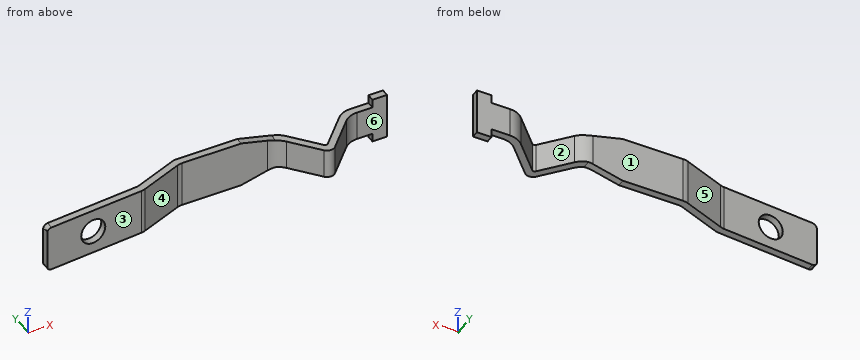
```python
from build123d import *

# Parameters (mm, degrees)
BOSS_EXTRUDE1_DEPTH = 4.75
SKETCH2_OUTSIDE_W   = 89.832
SKETCH2_OUTSIDE_H   = 26.332
SKETCH2_OUTSIDE_R   = 2.6
CUT_EXTRUDE1_DEPTH  = 30


with BuildPart() as part:
    # Sketch1 → Boss-Extrude1 (new, symmetric)
    with BuildSketch(Plane.XY):
        with BuildLine():
            Line((128.472093399, 20.626012941), (135.279511004, 20.626012941))
            Line((135.279511004, 20.626012941), (135.279511004, 19.126012941))
            Line((135.279511004, 19.126012941), (129.116456396, 19.126012941))
            ThreePointArc((129.116456396, 19.126012941), (127.537662704, 18.801255856), (126.215231232, 17.879718181))
            Line((126.215231232, 17.879718181), (120.723107444, 12.093373476))
            ThreePointArc((120.723107444, 12.093373476), (119.592910743, 11.626607721), (118.490782391, 12.156256613))
            Line((118.490782391, 12.156256613), (113.782718692, 17.712029816))
            ThreePointArc((113.782718692, 17.712029816), (112.412732854, 18.755342597), (110.731077047, 19.126012941))
            Line((110.731077047, 19.126012941), (93.127493614, 19.126012941))
            ThreePointArc((93.127493614, 19.126012941), (92.571949476, 19.074126018), (92.035622322, 18.920260082))
            Line((92.035622322, 18.920260082), (83.526071058, 15.595094388))
            ThreePointArc((83.526071058, 15.595094388), (83.117810035, 15.468266897), (82.695666994, 15.400757434))
            Line((82.695666994, 15.400757434), (62.410244618, 13.626012941))
            Line((62.410244618, 13.626012941), (62.279511004, 15.120304988))
            Line((62.279511004, 15.120304988), (82.350355756, 16.876276372))
            ThreePointArc((82.350355756, 16.876276372), (82.772498797, 16.943785835), (83.180759819, 17.070613325))
            Line((83.180759819, 17.070613325), (91.752961452, 20.420260082))
            ThreePointArc((91.752961452, 20.420260082), (92.289288606, 20.574126018), (92.844832744, 20.626012941))
            Line((92.844832744, 20.626012941), (111.42610449, 20.626012941))
            ThreePointArc((111.42610449, 20.626012941), (113.107760296, 20.255342597), (114.477746134, 19.212029816))
            Line((114.477746134, 19.212029816), (119.274777803, 13.551269534))
            ThreePointArc((119.274777803, 13.551269534), (119.64215392, 13.374719903), (120.018886154, 13.530308488))
            Line((120.018886154, 13.530308488), (125.570868236, 19.379718181))
            ThreePointArc((125.570868236, 19.379718181), (126.893299708, 20.301255856), (128.472093399, 20.626012941))
        make_face()
    extrude(amount=BOSS_EXTRUDE1_DEPTH, both=True)

    # Sketch2 outside → Cut-Extrude1 (cut)
    # profile 1 of 2: a face of its own
    with BuildSketch(Plane(origin=(0, 0, 0), x_dir=(1, 0, 0), z_dir=(0, 1, 0))):
        with Locations((98.78, 0)):
            Rectangle(SKETCH2_OUTSIDE_W, SKETCH2_OUTSIDE_H)
        with BuildLine():
            Line((132.279511004, 4.75), (132.279511004, 3))
            Line((132.279511004, 3), (112.256897869, 3))
            Line((112.256897869, 3), (105.256897869, 4.75))
            Line((105.256897869, 4.75), (63.279511004, 4.75))
            ThreePointArc((63.279511004, 4.75), (62.572404223, 4.457106781), (62.279511004, 3.75))
            Line((62.279511004, 3.75), (62.279511004, -3.75))
            ThreePointArc((62.279511004, -3.75), (62.572404223, -4.457106781), (63.279511004, -4.75))
            Line((63.279511004, -4.75), (105.256897869, -4.75))
            Line((105.256897869, -4.75), (112.256897869, -3))
            Line((112.256897869, -3), (132.279511004, -3))
            Line((132.279511004, -3), (132.279511004, -4.75))
            Line((132.279511004, -4.75), (135.279511004, -4.75))
            Line((135.279511004, -4.75), (135.279511004, 4.75))
            Line((135.279511004, 4.75), (132.279511004, 4.75))
        make_face(mode=Mode.SUBTRACT)
    # profile 2 of 2: a face of its own
    with BuildSketch(Plane(origin=(0, 0, 0), x_dir=(1, 0, 0), z_dir=(0, 1, 0))):
        with Locations(Location((72.279511004, 0, 0), (0, 0, 180))):
            Circle(SKETCH2_OUTSIDE_R)
    extrude(amount=CUT_EXTRUDE1_DEPTH, mode=Mode.SUBTRACT)


solid = part.part
```
The listing builds one solid part. Answer for the finished solid, in the listing's coordinates (mm). Face numbers are marked on the shaded views. A direction names the side the tool comes from. Give positions to 0.01 mm unless a question says otherwise; leave off trailing zeros. Order: outer loops, then holes, each group sorted by start corner. A loop starts at its lowest first (then second) coordinate and runs counter-clockwise, first axis right, second up. Notation, with made-up numbers: M -25.5,75.5 L 22.5,75.5 A18 cw 22.5,108.5 Z; hole C -7,77 d4. An arc over 180 degrees is marked long. Put each result on its own line as item: value. Start each with the question number.
Item 1: The part is cut by section B-B, the plane x = 74. Determine the outline of the cut face in (y, z), and give its area (3 significant figures).
Item 2: For a pull along X with two mould halves and no side action, classify the marked faces 4, 5 and 6 as +X half, -X half, draft (parallel to the pull), parting line (faces both ways), or undercut.
Item 3: Which of the six approach directions +Z, -Z, +X, -X, +Y, -Y give full straight-line access (tool end or side, diameter ignored) to the marked faces 1, 2 and 3?
Item 4: Flat-ended cylindrical pins translate along their axes: P1, Ø5, axis at x = 82, y = 17.5, coming from the -Z side; P2, Ø1.5, axis at x = 126.5, z = 1, coming from the +Y side; P3, Ø4.5, axis at x = 126, y = 16.5, coming from the -Z side; P4, Ø3, axis at x = 100, z = 1.5, coming from the -Y side. Find the tip coordinate at first contact, or state that the pin passes through.
Item 5: Find the intervals of material crossed by line 1 along X through (y, z) = (14.5, 0); line 2 along Y through (x, z) = (101, 1.5); line 3 along Z through (x, y) = (131, 19.5), in increasing order.
Item 6: The part is cut by section A-A, the plane z = 0. Determine the outline of the cut face in (x, y).
Item 7: The part is cut by section D-D, the plane x = 124.5. Determine the outline of the cut face in (y, z), and give its area (3 significant figures).
Item 8: The part is cut by section C-C, the plane x = 96.5. Determine the outline of the cut face in (y, z), and give its area (4 significant figures).
Answer key:
1. outline: M 14.64,-4.75 L 16.15,-4.75 L 16.15,-1.95 L 14.64,-1.95 Z; M 14.64,1.95 L 16.15,1.95 L 16.15,4.75 L 14.64,4.75 Z
1. area: 8.43 mm²
2. face 4: undercut
2. face 5: -X half
2. face 6: draft
3. face 1: +Z, -Z, +X, -X, +Y
3. face 2: +Z, -Z, +Y
3. face 3: +Z, -Z, -Y
4. P1: stops at z = -4.75
4. P2: stops at y = 20.43
4. P3: stops at z = -3
4. P4: stops at y = 19.13
5. line 1: x = 62.33 to 69.68, 116.5 to 118.47, 120.94 to 123.01
5. line 2: y = 19.13 to 20.63
5. line 3: z = -3 to 3
6. outline: M 62.28,15.12 L 62.41,13.63 L 69.68,14.26 L 69.68,15.77 Z; M 74.88,14.72 L 82.7,15.4 A3 ccw 83.53,15.6 L 92.04,18.92 A3 cw 93.13,19.13 L 110.73,19.13 A4 cw 113.78,17.71 L 118.49,12.16 A1.5 ccw 120.72,12.09 L 126.22,17.88 A4 cw 129.12,19.13 L 135.28,19.13 L 135.28,20.63 L 128.47,20.63 A4 ccw 125.57,19.38 L 120.02,13.53 A0.5 cw 119.27,13.55 L 114.48,19.21 A4 ccw 111.43,20.63 L 92.84,20.63 A3 ccw 91.75,20.42 L 83.18,17.07 A3 cw 82.35,16.88 L 74.88,16.22 Z
7. outline: M 16.07,-3 L 18.25,-3 L 18.25,3 L 16.07,3 Z
7. area: 13.1 mm²
8. outline: M 19.13,-4.75 L 20.63,-4.75 L 20.63,4.75 L 19.13,4.75 Z
8. area: 14.25 mm²
